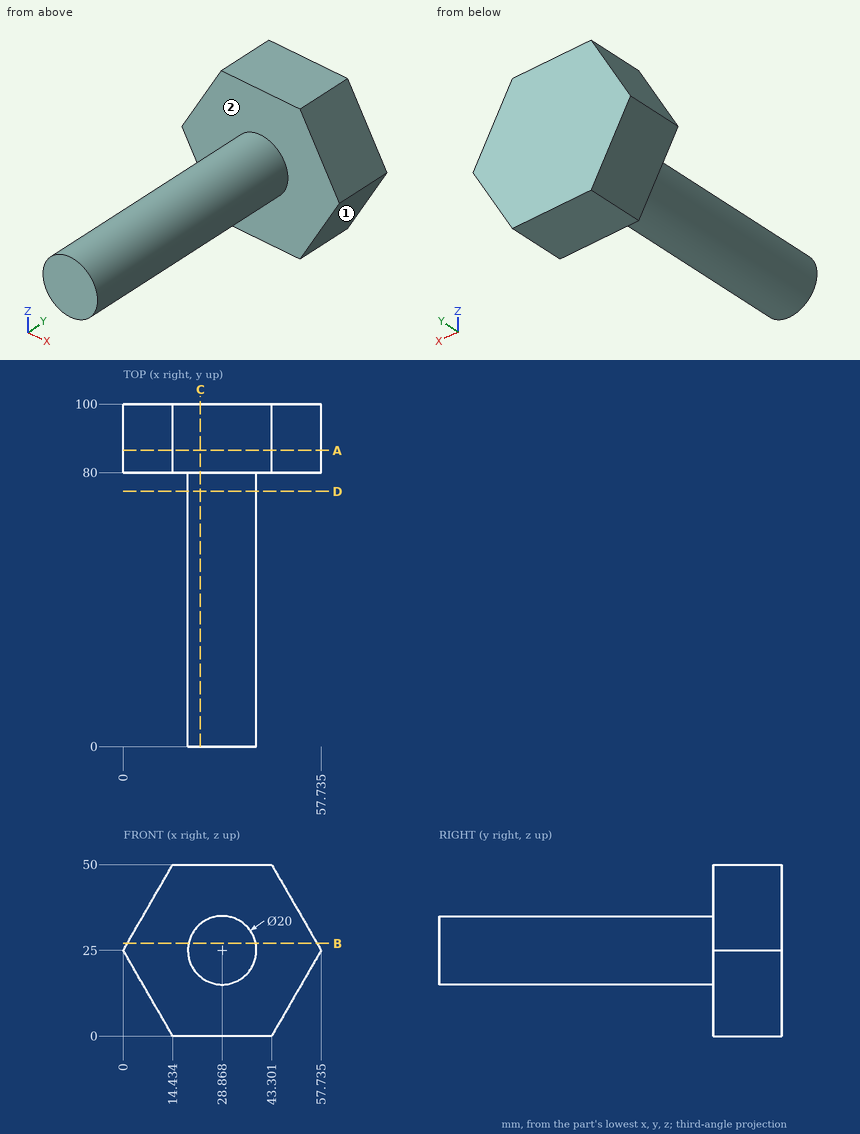
Part print with two shaded views. Sizes in mm from the minimum x, y, z corner. A direction names the side the tool comes from. Round coordinates to 2 decimals unless told otherwise and drop trailing zeros. Order: outer loops, then holes, each group sorted by start corner. A loop starts at its lowest first (then second) coordinate and runs counter-clockwise, first axis right, second up. Notation, with made-up numbers: (-36.5, 70) -> (-14.5, 70) arc R11 ccw to (-14.5, 91) -> close; hole circle Ø9 at (57.5, -18). An arc over 180 degrees is marked (long way). One line per question, with ' | ' between items.
Q1. Slice it at D-D (y = 74.5). Write the cut outline in (x, z), then the cut area to 3 significant figures.
Completed:
outline: circle Ø20 at (28.87, 25) | area: 314 mm^2
Q2. Slice it at B-B (z = 27). Write the cut outline in (x, y) (1 decimal), then the cut area to 3 significant figures.
Completed:
outline: (1.2, 80) -> (19.1, 80) -> (19.1, 0) -> (38.7, 0) -> (38.7, 80) -> (56.6, 80) -> (56.6, 100) -> (1.2, 100) -> close | area: 2,680 mm^2
Q3. Slice it at C-C (x = 22.5). Write the cut outline in (y, z), then the cut area to 3 significant figures.
Completed:
outline: (0, 17.29) -> (80, 17.29) -> (80, 0) -> (100, 0) -> (100, 50) -> (80, 50) -> (80, 32.71) -> (0, 32.71) -> close | area: 2,230 mm^2
Q4. Slice it at A-A (y = 86.5). Write the cut outline in (x, z) (1 decimal).
Completed:
outline: (0, 25) -> (14.4, 0) -> (43.3, 0) -> (57.7, 25) -> (43.3, 50) -> (14.4, 50) -> close
Q5. Probe probe 1 along Y at (x, z) = (6.5, 19.5); probe 2 along X at (y, z) = (48.5, 29.5); probe 3 along Z at (x, y) = (24, 12.5) (1 decimal). List the from-to ranges inside material, lowest first.
Completed:
probe 1: y = 80 to 100 | probe 2: x = 19.94 to 37.8 | probe 3: z = 16.3 to 33.7
Q6. Which spindle directions (+Z, -Z, +X, -X, +Y, -Y) get a long thin tool onto all of the face, cutting with end or side? Do the marked faces 1 and 2. Say none if no direction does.
Completed:
face 1: -Z, +X, +Y, -Y | face 2: -Y
Q7. Drop flat-ended pins along their axis: pin 1 (4 mm diameter, centred on y = 52, z = 27.5, fed in from -X); pin 2 (6 mm diameter, centred on x = 37, z = 11.5, fed in from -Y); pin 3 (4 mm diameter, centred on x = 18, y = 38.5, fed in from -Z) (1 decimal). Give the stop position or say it passes through.
Completed:
pin 1: stops at x = 18.88 | pin 2: stops at y = 80 | pin 3: stops at z = 20.4
